Can you work these out from the model? Positions are in its coordinate system, mm. A direction names the side the tool comes from. Give positions to 0.01 mm unless a question says otherwise; leave off trailing zeros. Order: outer loops, then holes, each group sorted by start corner. A loop starts at its lowest first (then second) coordinate and runs counter-clockwise, first axis right, second up. Notation, with made-up numbers: (26, 78) - (47, 78) arc R20 cw to (47, 100) - close; hole circle Ø7 at (-23.5, -36). An arc over 180 degrees is marked (long way). Return JSON: item names as keys, results as strings.
```python
from build123d import *

# Parameters (mm, degrees)
SKETCH_1_W                   = 115
SKETCH_1_H                   = 115
EXTRUDE_1_DEPTH              = 20
CUT_EXTRUDE_1_DEPTH          = 6
SKETCH_3_R                   = 32
CUT_EXTRUDE_2_DEPTH          = 84.740671122
SKETCH_4_R                   = 36
CUT_EXTRUDE_3_DEPTH          = 17
SKETCH_5_W                   = 11
SKETCH_5_H                   = 15.5
CUT_EXTRUDE_4_DEPTH          = 84.740671122
SKETCH_6_R                   = 2
CUT_EXTRUDE_5_DEPTH          = 84.740671122
HOLE_WIZARD_M6_1_D           = 6.6
HOLE_WIZARD_M6_1_CSINK_D     = 12.6
HOLE_WIZARD_M6_1_CSINK_ANGLE = 90
FILLET_1_R                   = 5
HOLE_WIZARD_M6_1_2_D         = 5
HOLE_WIZARD_M6_1_2_DEPTH     = 17
HOLE_WIZARD_M6_1_2_TIP       = 1.502151548
HOLE_WIZARD_M6_2_D           = 5
HOLE_WIZARD_M6_2_DEPTH       = 17
HOLE_WIZARD_M6_2_TIP         = 1.502151548


with BuildPart() as part:
    # 草图1 → 凸台-拉伸1 (new body)
    with BuildSketch(Plane.XY):
        Rectangle(SKETCH_1_W, SKETCH_1_H)
    extrude(amount=EXTRUDE_1_DEPTH)

    # 草图2 → 切除-拉伸1 (cut)
    with BuildSketch(Plane(origin=(0, 0, 0), x_dir=(-1, 0, 0), z_dir=(0, 0, -1))):
        Polygon((-57.5, 57.5), (-42.5, 57.5), (-42.5, -42.5), (57.5, -42.5), (57.5, -57.5), (-57.5, -57.5), align=None)
    extrude(amount=-CUT_EXTRUDE_1_DEPTH, mode=Mode.SUBTRACT)

    # 草图3 → 切除-拉伸2 (cut, through all)
    with BuildSketch(Plane(origin=(0, 0, 0), x_dir=(-1, 0, 0), z_dir=(0, 0, -1))):
        with Locations((17.5, 17.5)):
            Circle(SKETCH_3_R)
    extrude(amount=-CUT_EXTRUDE_2_DEPTH, mode=Mode.SUBTRACT)

    # 草图4 → 切除-拉伸3 (cut)
    with BuildSketch(Plane(origin=(0, 0, 0), x_dir=(-1, 0, 0), z_dir=(0, 0, -1))):
        with Locations((17.5, 17.5)):
            Circle(SKETCH_4_R)
    extrude(amount=-CUT_EXTRUDE_3_DEPTH, mode=Mode.SUBTRACT)

    # 草图5 → 切除-拉伸4 (cut, through all)
    with BuildSketch(Plane.XY.offset(20)):
        with Locations((-0.5, -49.75)):
            Rectangle(SKETCH_5_W, SKETCH_5_H)
    extrude(amount=-CUT_EXTRUDE_4_DEPTH, mode=Mode.SUBTRACT)

    # 草图6 → 切除-拉伸5 (cut, through all)
    with BuildSketch(Plane.XY.offset(20)):
        with Locations((-6, -42)):
            Circle(SKETCH_6_R)
        with Locations((5, -42)):
            Circle(SKETCH_6_R)
    extrude(amount=-CUT_EXTRUDE_5_DEPTH, mode=Mode.SUBTRACT)

    # Hole Wizard M6 _1 (through all)
    with Locations(Plane.XY.offset(20)):
        with Locations((-37.5, -50), (22.5, -50), (50, -22.5), (50, 37.5)):
            CounterSinkHole(HOLE_WIZARD_M6_1_D / 2, HOLE_WIZARD_M6_1_CSINK_D / 2, counter_sink_angle=HOLE_WIZARD_M6_1_CSINK_ANGLE)

    # 圆角1
    fillet_1_edges = [part.edges().sort_by_distance(p)[0] for p in [
        (-57.5, 57.5, 10),
    ]]
    fillet(fillet_1_edges, radius=FILLET_1_R)

    # Hole Wizard M6 _1 2
    with Locations(Plane.XY.offset(20)):
        with Locations((32.5, 45.5), (14.5, 45.5)):
            Hole(HOLE_WIZARD_M6_1_2_D / 2, depth=HOLE_WIZARD_M6_1_2_DEPTH)
            with Locations((0, 0, -(HOLE_WIZARD_M6_1_2_DEPTH + HOLE_WIZARD_M6_1_2_TIP / 2))):  # 118° drill point
                Cone(0, HOLE_WIZARD_M6_1_2_D / 2, HOLE_WIZARD_M6_1_2_TIP, mode=Mode.SUBTRACT)

    # M6 螺纹孔2
    with Locations(Plane(origin=(0, 57.5, 0), x_dir=(1, 0, 0), z_dir=(0, 1, 0))):
        with Locations((-42.5, -10), (12.5, -10)):
            Hole(HOLE_WIZARD_M6_2_D / 2, depth=HOLE_WIZARD_M6_2_DEPTH)
            with Locations((0, 0, -(HOLE_WIZARD_M6_2_DEPTH + HOLE_WIZARD_M6_2_TIP / 2))):  # 118° drill point
                Cone(0, HOLE_WIZARD_M6_2_D / 2, HOLE_WIZARD_M6_2_TIP, mode=Mode.SUBTRACT)


solid = part.part
```
1. Suppose I cut it at B-B (y = -50). List the corners of the cut face in (x, z) for me, plus the area to 3 significant figures.
Checks:
{"outline": "(-57.5, 6) - (-40.8, 6) - (-40.8, 17) - (-43.8, 20) - (-57.5, 20) - close; (-34.2, 6) - (-6, 6) - (-6, 20) - (-31.2, 20) - (-34.2, 17) - close; (5, 6) - (19.2, 6) - (19.2, 17) - (16.2, 20) - (5, 20) - close; (25.8, 6) - (57.5, 6) - (57.5, 20) - (28.8, 20) - (25.8, 17) - close", "area": "1,250 mm^2"}
2. Suppose I cut it at D-D (z = 14.5). List the corners of the cut face in (x, y) for me.
Checks:
{"outline": "(-57.5, -57.5) - (-6, -57.5) - (-6, -44) arc R2 cw (long way) to (-4, -42) - (3, -42) arc R2 cw (long way) to (5, -44) - (5, -57.5) - (57.5, -57.5) - (57.5, 57.5) - (-52.5, 57.5) arc R5 ccw to (-57.5, 52.5) - close; hole circle Ø72 at (-17.5, 17.5); hole circle Ø6.6 at (-37.5, -50); hole circle Ø5 at (14.5, 45.5); hole circle Ø6.6 at (22.5, -50); hole circle Ø5 at (32.5, 45.5); hole circle Ø6.6 at (50, -22.5); hole circle Ø6.6 at (50, 37.5)"}
3. Suppose I cut it at A-A (x = -17.5). List the corners of the cut face in (y, z) for me, plus the area to 3 significant figures.
Checks:
{"outline": "(-57.5, 6) - (-42.5, 6) - (-42.5, 0) - (-18.5, 0) - (-18.5, 17) - (-14.5, 17) - (-14.5, 20) - (-57.5, 20) - close; (49.5, 17) - (53.5, 17) - (53.5, 0) - (57.5, 0) - (57.5, 20) - (49.5, 20) - close", "area": "794 mm^2"}
4. On a 3-axis mill with a long thin cutter (end or side, diameter ignored), from which of +Z, -Z, +X, -X, +Y, -Y can I reach the whole of each face in a straight line? I mean faces 4 (the face through (-44.81, 50.86, 10.96)), 5 (the face through (-32, -42.5, 3)), 6 (the face through (11.068, -4.405, 8.381)), 7 (the face through (42.5, 8, 3)). Say none if no direction works.
Checks:
{"face 4": "+Y", "face 5": "-Z, +X, -X, -Y", "face 6": "-Z", "face 7": "-Z, +X, +Y, -Y"}
5. Suppose I cut it at C-C (y = 17.5). List the corners of the cut face in (x, z) for me.
Checks:
{"outline": "(-57.5, 0) - (-53.5, 0) - (-53.5, 17) - (-49.5, 17) - (-49.5, 20) - (-57.5, 20) - close; (14.5, 17) - (18.5, 17) - (18.5, 0) - (42.5, 0) - (42.5, 6) - (57.5, 6) - (57.5, 20) - (14.5, 20) - close"}
6. For pin 1 Ø12 at (x, y) = (-11, 41.5) entering from -Z; pin 2 Ø1.8 at (x, z) = (-45, 3.5) entering from -Y; pin 3 Ø3 at (x, y) = (32.5, 45.5) entering from +Z; pin 4 Ø1.5 at (y, z) = (16.5, 3.5) entering from +X, each with a flat end and sliding along its axis, tell me the tip position at first contact or that it passes through.
Checks:
{"pin 1": "through", "pin 2": "y = -42.5", "pin 3": "z = 2.4", "pin 4": "x = 42.5"}
7. If I drill on L1, parallel to Y at x = -17.5, z = 18.1; L2, parallel to X at y = 45.5, z = 7.75; L3, parallel to Y at x = 14.5, z = 14.75, over which ranges is the centre line in solid material (lowest first)? Write a range as [from, to].
Checks:
{"L1": "[-57.5, -14.5], [49.5, 57.5]", "L2": "[-57.5, -43.59], [-41.41, -40.13], [5.13, 11.41], [17, 30], [35, 57.5]", "L3": "[-57.5, 1.01], [33.99, 43], [48, 57.5]"}
8. Thinking about a two-plate mould opening in Z: for faces 1 (the face through (10.19, 48.88, 10.96)), 2 (the face through (7, -4, 17)), 3 (the face through (-56.07, 56, 10.14)), which applies, +Z half, -Z half, draft (parallel to the pull), parting line (faces both ways), or undercut?
Checks:
{"face 1": "undercut", "face 2": "-Z half", "face 3": "draft"}
